Here's how the part is built. I have some questions about the finished solid (model axes, mm). Face numbers are marked on the shaded views. A direction names the side the tool comes from. Round coordinates to 2 decimals unless told otherwise and drop trailing zeros. Write each loop counter-clockwise with the first axis right and the second up, starting at its lowest first coordinate (ties: lowest second). Pieces come first, ordered by that corner, then holes. Notation, with made-up numbers: (-37, -10) - (-33, -10) arc R27 cw to (-33, 24) - close; hole circle Ø1 at (84.25, -19.75). An arc over 180 degrees is marked (long way). Use one line per item in the form item = value. Start each with the question number.
1. Which directions (+Z, -Z, +X, -X, +Y, -Y) give clear straight access to the entire face, cutting with the end or side of a thin tool? Please do the marked faces 1, 2 and 3.
2. I want a section at B-B, the plane x = 17.78. List the corners of the cut face in (y, z) for me, plus the area to 3 significant figures.
3. I want a section at A-A, the plane y = 11.5. List the corners of the cut face in (x, z) for me (3 decimals).
4. Will this pin go through, and if not, where does the flat tip stop? pin 1 (4 mm diameter, centred on y = 11.5, z = 17, fed in from -X).
5. If I drill on line 1 along Z through (x, y) = (-17.78, -28.75); line 2 along Y through (x, z) = (-12, 34); line 3 along X through (y, z) = (-20, 5.5), over which ranges is the centre line in solid material (lowest first)?
6. I want a section at D-D, the plane z = 19.5. List the corners of the cut face in (x, y) for me.
7. We'd pull the mould along X, two halves only. Please class the marked faces 4, 5, 6 and 7: +X half, -X half, draft (parallel to the pull), parting line (faces both ways), or undercut.
8. I want a section at C-C, the plane y = -7.5. List the corners of the cut face in (x, z) for me (3 decimals).
```python
from build123d import *

# Parameters (mm, degrees)
BLOCK_PROFILE_SKETCH_W  = 76.2
BLOCK_PROFILE_SKETCH_H  = 76.2
BLOCK_BODY_3IN_DEPTH    = 38.1
ANGLED_SLOT_CUT_DEPTH   = 10.16
SLOT_UNDERCUT_CUT_DEPTH = 20.32
EDGE_FILLETS_R0_125_R   = 3.175
TOP_HOLES_SKETCH_R      = 6.35
TOP_HOLES_SKETCH_R_2    = 12.7
TOP_HOLES_3X_DEPTH      = 94.3255592


with BuildPart() as part:
    # Block Profile Sketch → Block Body 3in (new, symmetric)
    with BuildSketch(Plane.XY):
        Rectangle(BLOCK_PROFILE_SKETCH_W, BLOCK_PROFILE_SKETCH_H)
    extrude(amount=BLOCK_BODY_3IN_DEPTH, both=True)

    # Angled Slot Sketch → Angled Slot Cut (cut)
    with BuildSketch(Plane.ZY.offset(38.1)):
        Polygon((38.1, -17.24611593), (-38.1, -3.81), (-38.1, 19.05), (38.1, 19.05), align=None)
    extrude(amount=-ANGLED_SLOT_CUT_DEPTH, mode=Mode.SUBTRACT)

    # Slot Undercut Sketch → Slot Undercut Cut (cut)
    with BuildSketch(Plane.ZY.offset(27.94)):
        Polygon((-38.1, 25.4), (38.1, 25.4), (38.1, -26.13611593), (-38.1, -12.7), align=None)
    extrude(amount=-SLOT_UNDERCUT_CUT_DEPTH, mode=Mode.SUBTRACT)

    # Edge Fillets R0.125
    edge_fillets_r0_125_edges = [part.edges().sort_by_distance(p)[0] for p in [
        (-38.1, 28.575, 38.1),
        (-38.1, -20.955, -38.1),
        (-38.1, -27.673057965, 38.1),
        (38.1, 0, 38.1),
        (-38.1, 28.575, -38.1),
        (38.1, 0, -38.1),
    ]]
    fillet(edge_fillets_r0_125_edges, radius=EDGE_FILLETS_R0_125_R)

    # Top Holes Sketch → Top Holes 3x (cut, through all)
    with BuildSketch(Plane(origin=(0, 38.1, 0), x_dir=(1, 0, 0), z_dir=(0, 1, 0))):
        with Locations(Location((-17.78, 19.05, 0), (0, 0, 270))):
            Circle(TOP_HOLES_SKETCH_R)
        with Locations(Location((-17.78, -19.05, 0), (0, 0, 270))):
            Circle(TOP_HOLES_SKETCH_R)
        with Locations(Location((17.78, 0, 0), (0, 0, 270))):
            Circle(TOP_HOLES_SKETCH_R_2)
    extrude(amount=-TOP_HOLES_3X_DEPTH, mode=Mode.SUBTRACT)


solid = part.part
```
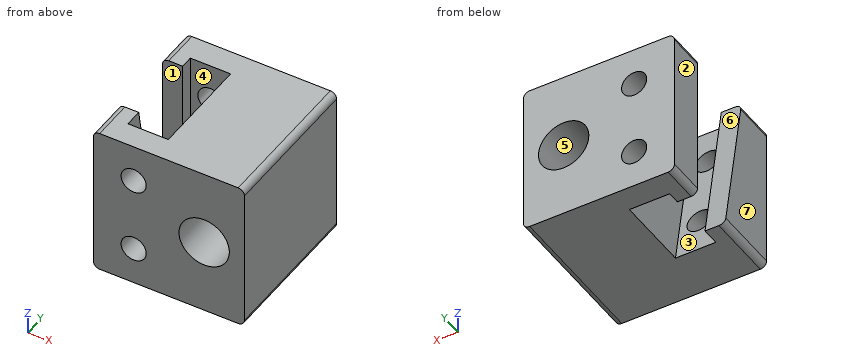
Model answer:
q1.face_1 = +Z, -Z, -X
q1.face_2 = +Z, -Z, -X, +Y, -Y
q1.face_3 = +Z
q2.outline = (-38.1, -38.1) - (38.1, -38.1) - (38.1, -12.7) - (-38.1, -12.7) - close; (-38.1, 12.7) - (38.1, 12.7) - (38.1, 38.1) - (-38.1, 38.1) - close
q2.area = 3,870 mm2
q3.outline = (-7.62, -38.1) - (34.925, -38.1) arc R3.175 ccw to (38.1, -34.925) - (38.1, 34.925) arc R3.175 ccw to (34.925, 38.1) - (-7.62, 38.1) - close; hole circle Ø25.4 at (17.78, 0)
q4.pin_1 = -7.62
q5.line_1 = -38.1 to -25.4, -12.7 to 12.7, 25.4 to 38.1
q5.line_2 = -38.1 to -25.41, 25.4 to 38.1
q5.line_3 = -38.1 to -27.94, -7.62 to 6.33, 29.23 to 38.1
q6.outline = (-38.1, -38.1) - (-24.11, -38.1) - (-24.11, -22.86) - (-27.94, -22.86) - (-27.94, -13.97) - (-38.1, -13.97) - close; (-38.1, 19.05) - (-27.94, 19.05) - (-27.94, 25.4) - (-24.11, 25.4) - (-24.11, 38.1) - (-38.1, 38.1) - close; (-11.45, -38.1) - (38.1, -38.1) - (38.1, 38.1) - (-11.45, 38.1) - (-11.45, 25.4) - (-7.62, 25.4) - (-7.62, -22.86) - (-11.45, -22.86) - close
q7.face_4 = undercut
q7.face_5 = undercut
q7.face_6 = draft
q7.face_7 = -X half
q8.outline = (-38.1, -34.925) arc R3.175 ccw to (-34.925, -38.1) - (-27.94, -38.1) - (-27.94, -17.173) - (-38.1, -17.173) - close; (-7.62, -38.1) - (34.925, -38.1) arc R3.175 ccw to (38.1, -34.925) - (38.1, 34.925) arc R3.175 ccw to (34.925, 38.1) - (-7.62, 38.1) - close; hole circle Ø25.4 at (17.78, 0)
